from build123d import *

# Parameters (mm, degrees)
C_FRAME_DEPTH         = 22.5
FRONT_POCKET_DEPTH    = 7.5
BACK_START            = -7.5
BACK_POCKET_DEPTH     = 7.5
SCREW_BOSS_DEPTH      = 18.5
SCREW_BOSS_DEPTH_BACK = 58.5
SCREW_BOSS_SKETCH_R   = 22.5
SCREW_HOLE_SKETCH_R   = 10
SCREW_HOLE_DEPTH      = 98.5


with BuildPart() as part:
    # C Frame Profile Sketch → C Frame (new, symmetric)
    with BuildSketch(Plane.XY):
        with BuildLine():
            Line((108.518716773, 232), (-30.481283227, 238.150273432))
            Line((-30.481283227, 238.150273432), (-30.481283227, 24.391710358))
            ThreePointArc((-30.481283227, 24.391710358), (-21.101269131, 4.872078181), (0, 0))
            Line((0, 0), (89, 20))
            ThreePointArc((89, 20), (103.038348951, 28.771724453), (108.518716773, 44.391710358))
            Line((108.518716773, 44.391710358), (108.518716773, 67))
            Line((108.518716773, 67), (58.518716773, 67))
            ThreePointArc((58.518716773, 67), (40.841047244, 74.32233047), (33.518716773, 92))
            Line((33.518716773, 92), (33.518716773, 192))
            Line((33.518716773, 192), (108.518716773, 192))
            Line((108.518716773, 192), (108.518716773, 232))
        make_face()
    extrude(amount=C_FRAME_DEPTH, both=True)

    # Front Pocket Sketch → Front Pocket (cut)
    with BuildSketch(Plane.XY.offset(22.5)):
        with BuildLine():
            Line((-22.481283227, 229.788473653), (-22.481283227, 24.391710358))
            ThreePointArc((-22.481283227, 24.391710358), (-16.102873642, 11.118360478), (-1.754010632, 7.805347315))
            Line((-1.754010632, 7.805347315), (87.245989368, 27.805347315))
            ThreePointArc((87.245989368, 27.805347315), (96.792066654, 33.770119943), (100.518716773, 44.391710358))
            Line((100.518716773, 44.391710358), (100.518716773, 59))
            Line((100.518716773, 59), (58.518716773, 59))
            ThreePointArc((58.518716773, 59), (35.184192994, 68.665476221), (25.518716773, 92))
            Line((25.518716773, 92), (25.518716773, 200))
            Line((25.518716773, 200), (85.464789993, 200))
            ThreePointArc((85.464789993, 200), (97.961735105, 212.223661697), (86.017331529, 224.987781943))
            Line((86.017331529, 224.987781943), (-22.481283227, 229.788473653))
        make_face()
    extrude(amount=-FRONT_POCKET_DEPTH, mode=Mode.SUBTRACT)

    # Back Pocket Sketch → Back Pocket (cut)
    with BuildSketch(Plane(origin=(0, 0, -22.5), x_dir=(-1, 0, 0), z_dir=(0, 0, -1)).offset(BACK_START)):
        with BuildLine():
            Line((-58.518716773, 59), (-100.518716773, 59))
            Line((-100.518716773, 59), (-100.518716773, 44.391710358))
            ThreePointArc((-100.518716773, 44.391710358), (-96.792066654, 33.770119943), (-87.245989368, 27.805347315))
            Line((-87.245989368, 27.805347315), (1.754010632, 7.805347315))
            ThreePointArc((1.754010632, 7.805347315), (16.102873642, 11.118360478), (22.481283227, 24.391710358))
            Line((22.481283227, 24.391710358), (22.481283227, 229.788473653))
            Line((22.481283227, 229.788473653), (-100.518716773, 224.346145364))
            Line((-100.518716773, 224.346145364), (-100.518716773, 200))
            Line((-100.518716773, 200), (-25.518716773, 200))
            Line((-25.518716773, 200), (-25.518716773, 92))
            ThreePointArc((-25.518716773, 92), (-35.184192994, 68.665476221), (-58.518716773, 59))
        make_face()
    extrude(amount=BACK_POCKET_DEPTH, mode=Mode.SUBTRACT)

    # Screw Boss Sketch → Screw Boss (add, two sides: drawn at the far end of the back side and taken through both)
    with BuildSketch(Plane(origin=(10.457185431, 236.338886554, 0), x_dir=(0.9990225554240701, -0.0442033228837011, 0), z_dir=(0.0442033228837011, 0.9990225554240703, 0)).offset(-SCREW_BOSS_DEPTH_BACK)):
        with Locations(Location((82.951023109, 0, 0), (0, 0, 180))):
            Circle(SCREW_BOSS_SKETCH_R)
    extrude(amount=SCREW_BOSS_DEPTH + SCREW_BOSS_DEPTH_BACK)

    # Screw Hole Sketch → Screw Hole (cut)
    with BuildSketch(Plane(origin=(11.274946905, 254.820803829, 0), x_dir=(0.9990225554240701, -0.04420332288370111, 0), z_dir=(0.04420332288370111, 0.9990225554240703, 0))):
        with Locations(Location((82.951023109, 0, 0), (0, 0, 180))):
            Circle(SCREW_HOLE_SKETCH_R)
    extrude(amount=-SCREW_HOLE_DEPTH, mode=Mode.SUBTRACT)


solid = part.part
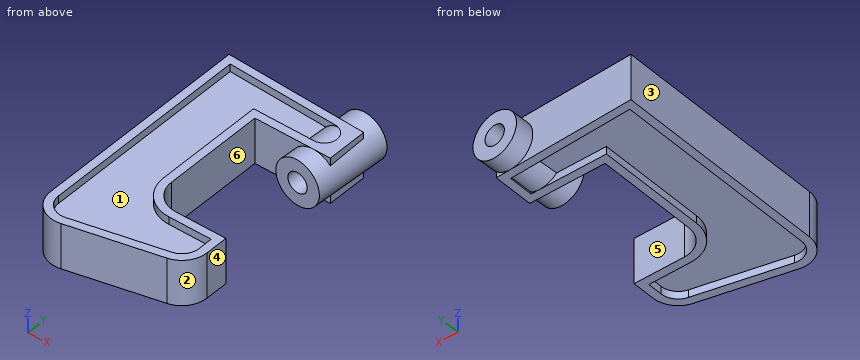
For this review, take the finished solid that the model builds, in its own axes (mm). Face numbers are marked on the shaded views. A direction names the side the tool comes from. Give positions to 0.01 mm unless a question says otherwise; leave off trailing zeros. Loops run counter-clockwise (first coordinate to the right, second up) from the corner with the lowest first, then second, coordinate; pieces in that order, holes last.
Item 1: Take a section at B-B, the plane y = 136. State the section outline as (x, z) points, and give its area (3 significant figures).
Item 2: Insertion check: pin 1 (4 mm diameter, centred on x = 5.5, y = 158.5, fed in from +Z); pin 2 (8 mm diameter, centred on x = 83, z = 19.5, fed in from -Y); pin 3 (18 mm diameter, centred on y = 53.5, z = 10.5, fed in from +X); pin 4 (2 mm diameter, centred on x = 64, y = 68.5, fed in from -Z). Each pin has a flat end and moves straight along its axis. Give the tip position at first contact, or say it passes through.
Item 3: Tool access review of the marked faces 4, 5 and 6: name each direction out of +Z, -Z, +X, -X, +Y, -Y from which nothing blocks a thin tool from reaching the whole face with its end or side.
Item 4: For line 1 along Y through (x, z) = (40, -16); line 2 along X through (y, z) = (196.5, -16); line 3 along X through (y, z) = (45.5, 18), list the stretches that pass through material, from the lowest coordinate up.
Item 5: Take a section at A-A, the plane x = 54.5. State the section outline as (y, z) points, and give its area (3 significant figures).
Item 6: Draft analysis for pull direction X (two halves, no side actions). For the marked faces 1, 2 and 3, state which applies: +X half, -X half, draft (parallel to the pull), parting line (faces both ways), or undercut.
Item 7: Take a section at C-C, the plane z = 6. State the section outline as (x, y) points.
Calculated:
1. outline: (-30.48, -22.5) - (-22.48, -22.5) - (-22.48, -15) - (25.52, -15) - (25.52, -22.5) - (33.52, -22.5) - (33.52, 22.5) - (25.52, 22.5) - (25.52, 15) - (-22.48, 15) - (-22.48, 22.5) - (-30.48, 22.5) - close
1. area: 2,160 mm2
2. pin 1: stops at z = 15
2. pin 2: stops at y = 17.75
2. pin 3: stops at x = 108.52
2. pin 4: passes through
3. face 4: +Z, -Z, +X, -Y
3. face 5: +Z, -Z, +X
3. face 6: +Z, -Z
4. line 1: y = 8.99 to 17.19, 64.69 to 75.21, 192 to 200, 227.02 to 235.03
4. line 2: x = -30.48 to -22.48, 25.52 to 108.52
4. line 3: x = -30.48 to -22.48, 100.52 to 108.52
5. outline: (12.25, -22.5) - (20.45, -22.5) - (20.45, -15) - (59.25, -15) - (59.25, -22.5) - (67.33, -22.5) - (67.33, 22.5) - (59.25, 22.5) - (59.25, 15) - (20.45, 15) - (20.45, 22.5) - (12.25, 22.5) - close; (192, -22.5) - (200, -22.5) - (200, -15) - (226.38, -15) - (226.38, -22.5) - (234.39, -22.5) - (234.39, 22.5) - (226.38, 22.5) - (226.38, 15) - (200, 15) - (200, 22.5) - (192, 22.5) - close
5. area: 3,410 mm2
6. face 1: undercut
6. face 2: +X half
6. face 3: -X half
7. outline: (-30.48, 24.39) arc R25 ccw to (0, 0) - (89, 20) arc R25 ccw to (108.52, 44.39) - (108.52, 67) - (58.52, 67) arc R25 cw to (33.52, 92) - (33.52, 192) - (69.82, 192) - (69.08, 175.19) - (82.75, 174.58) - (86.15, 251.51) - (72.48, 252.11) - (71.66, 233.63) - (-30.48, 238.15) - close; (98.73, 173.88) - (112.41, 173.27) - (115.81, 250.2) - (102.14, 250.8) - close
